```python
from build123d import *

# Parameters (mm, degrees)
SKETCH1_W           = 350
SKETCH1_H           = 120
BOSS_EXTRUDE1_DEPTH = 25
SKETCH2_W           = 180
SKETCH2_H           = 20
CUT_EXTRUDE1_DEPTH  = 214.658606192
SKETCH3_R           = 11
CUT_EXTRUDE2_DEPTH  = 25
FILLET1_R           = 0.5


with BuildPart() as part:
    # Sketch1 → Boss-Extrude1 (new body)
    with BuildSketch(Plane(origin=(0, 0, 0), x_dir=(1, 0, 0), z_dir=(0, 1, 0))):
        Rectangle(SKETCH1_W, SKETCH1_H)
    extrude(amount=BOSS_EXTRUDE1_DEPTH)

    # Sketch2 → Cut-Extrude1 (cut, through all)
    with BuildSketch(Plane.XY.offset(60)):
        Rectangle(SKETCH2_W, SKETCH2_H)
    extrude(amount=-CUT_EXTRUDE1_DEPTH, mode=Mode.SUBTRACT)

    # Sketch3 → Cut-Extrude2 (cut)
    with BuildSketch(Plane(origin=(0, 25, 0), x_dir=(1, 0, 0), z_dir=(0, 1, 0))):
        with Locations(Location((-145, 0, 0), (0, 0, 270))):
            Circle(SKETCH3_R)
        with Locations(Location((145, 0, 0), (0, 0, 90))):
            Circle(SKETCH3_R)
    extrude(amount=-CUT_EXTRUDE2_DEPTH, mode=Mode.SUBTRACT)

    # Fillet1
    fillet1_edges = [part.edges().sort_by_distance(p)[0] for p in [
        (90, 10, 0),
        (-90, 10, 0),
    ]]
    fillet(fillet1_edges, radius=FILLET1_R)


solid = part.part
```
For this review, take the finished solid that the model builds, in its own axes (mm). A direction names the side the tool comes from. Round coordinates to 2 decimals unless told otherwise and drop trailing zeros. Order: outer loops, then holes, each group sorted by start corner. A loop starts at its lowest first (then second) coordinate and runs counter-clockwise, first axis right, second up. Notation, with made-up numbers: (45, 18.5) -> (68, 18.5) arc R8 cw to (68, 32.5) -> close; hole circle Ø11 at (-39, 38.25). An arc over 180 degrees is marked (long way). Use a Markdown table: item, result.
Item 1: For pin 1 (1 mm diameter, centred on x = -37.5, z = 48, fed in from -Y); pin 2 (17.5 mm diameter, centred on x = -145, z = 0, fed in from +Y), all flat-tipped, find the tip position at first contact; note any pin that passes through.
Resolved:
| item | result |
|---|---|
| pin 1 | stops at y = 10 |
| pin 2 | passes through |
Item 2: Take a section at B-B (z = 0). State the section outline as (x, y) points, plus the area to 3 significant figures.
Resolved:
| item | result |
|---|---|
| outline | (-175, 0) -> (-156, 0) -> (-156, 25) -> (-175, 25) -> close; (-134, 0) -> (-90, 0) -> (-90, 9.5) arc R0.5 cw to (-89.5, 10) -> (89.5, 10) arc R0.5 cw to (90, 9.5) -> (90, 0) -> (134, 0) -> (134, 25) -> (-134, 25) -> close; (156, 0) -> (175, 0) -> (175, 25) -> (156, 25) -> close |
| area | 5,850 mm² |
Item 3: For line 1 along X through (y, z) = (14.25, 0); line 2 along X through (y, z) = (7.5, 0); line 3 along Z through (x, y) = (145, 8.75), list the stretches that pass through material, from the lowest coordinate up. Write a range as [from, to].
Resolved:
| item | result |
|---|---|
| line 1 | x = [-175, -156], [-134, 134], [156, 175] |
| line 2 | x = [-175, -156], [-134, -90], [90, 134], [156, 175] |
| line 3 | z = [-60, -11], [11, 60] |
Item 4: Take a section at C-C (x = 145). State the section outline as (y, z) points, plus the area to 3 significant figures.
Resolved:
| item | result |
|---|---|
| outline | (0, -60) -> (25, -60) -> (25, -11) -> (0, -11) -> close; (0, 11) -> (25, 11) -> (25, 60) -> (0, 60) -> close |
| area | 2,450 mm² |
Item 5: Take a section at D-D (z = -21). State the section outline as (x, y) points.
Resolved:
| item | result |
|---|---|
| outline | (-175, 0) -> (-90, 0) -> (-90, 9.5) arc R0.5 cw to (-89.5, 10) -> (89.5, 10) arc R0.5 cw to (90, 9.5) -> (90, 0) -> (175, 0) -> (175, 25) -> (-175, 25) -> close |
Item 6: Take a section at A-A (y = 3.75). State the section outline as (x, z) points, plus the area to 3 significant figures.
Resolved:
| item | result |
|---|---|
| outline | (-175, -60) -> (-90, -60) -> (-90, 60) -> (-175, 60) -> close; (90, -60) -> (175, -60) -> (175, 60) -> (90, 60) -> close; hole circle Ø22 at (-145, 0); hole circle Ø22 at (145, 0) |
| area | 19,600 mm² |
Item 7: Machinability: for faces 1 (the flat face through (132, 0, -1)), 2 (the flat face through (-90, 5, 1)), which of the approach directions +Z, -Z, +X, -X, +Y, -Y give a long, thin tool a straight path to every point of the face, cutting with its end or side? Answer none if there is none.
Resolved:
| item | result |
|---|---|
| face 1 | +Z, -Z, +X, -X, -Y |
| face 2 | +Z, -Z, -Y |
Item 8: Draft analysis for pull direction X (two halves, no side actions). For faces 3 (the flat face through (-2, 25, -1)), 4 (the flat face through (175, 12, 1)), 5 (the flat face through (90, 5, 1)), state which applies: +X half, -X half, draft (parallel to the pull), parting line (faces both ways), or undercut.
Resolved:
| item | result |
|---|---|
| face 3 | draft |
| face 4 | +X half |
| face 5 | undercut |
